Verification items for the finished model (mm, model axes). A direction names the side the tool comes from. Coordinates: 2 decimals unless noted, no trailing zeros. Write each loop counter-clockwise with the first axis right and the second up, starting at its lowest first coordinate (ties: lowest second). Pieces come first, ordered by that corner, then holes. Notation, with made-up numbers: (10.25, 74) -> (30.25, 74) arc R9 cw to (30.25, 86) -> close; hole circle Ø8 at (36, -1.75). An arc over 180 degrees is marked (long way). Answer in a Markdown table with one row per item.
```python
from build123d import *

# Parameters (mm, degrees)
SKETCH1_R                  = 40
SKETCH1_R_2                = 30
BOSS_EXTRUDE1_DEPTH        = 537.5
CUT_EXTRUDE1_START         = -25
SKETCH2_R                  = 55.029082457
SKETCH2_R_2                = 36.75
CUT_EXTRUDE1_DEPTH         = 3
SKETCH3_R                  = 40
SKETCH3_R_2                = 38
CUT_EXTRUDE2_DEPTH         = 25
CHAMFER1_SIZE              = 1
SKETCH4_R                  = 33.575067705
BOSS_EXTRUDE2_DEPTH        = 40
SKETCH5_R                  = 25
CUT_EXTRUDE3_DEPTH         = 6
SKETCH6_R                  = 21.5
CUT_EXTRUDE4_DEPTH         = 535.501870904
CHAMFER2_SIZE              = 1
SKETCH9_R                  = 30
CUT_EXTRUDE7_DEPTH         = 40
SKETCH10_R                 = 35
CUT_EXTRUDE8_DEPTH         = 7
M64X4_0_TAPPED_HOLE1_D     = 60
M64X4_0_TAPPED_HOLE1_DEPTH = 20
M64X4_0_TAPPED_HOLE1_TIP   = 18.025818571
CHAMFER3_SIZE              = 0.5
CHAMFER4_SIZE              = 0.5
SKETCH13_R                 = 40
CUT_EXTRUDE9_DEPTH         = 3
CHAMFER5_SIZE              = 1
CHAMFER7_SIZE              = 0.5
FILLET1_R                  = 0.5
M64X3_0_TAPPED_HOLE1_D     = 61
M64X3_0_TAPPED_HOLE1_DEPTH = 55
M64X3_0_TAPPED_HOLE1_TIP   = 18.32624888
CHAMFER8_SIZE              = 1


with BuildPart() as part:
    # Sketch1 → Boss-Extrude1 (new body)
    with BuildSketch(Plane(origin=(0, 0, 0), x_dir=(1, 0, 0), z_dir=(0, 1, 0))):
        with Locations(Location((0, 0, 0), (0, 0, 270))):
            Circle(SKETCH1_R)
        with Locations(Location((0, 0, 0), (0, 0, 270))):
            Circle(SKETCH1_R_2, mode=Mode.SUBTRACT)
    extrude(amount=BOSS_EXTRUDE1_DEPTH)

    # Sketch2 → Cut-Extrude1 (cut)
    with BuildSketch(Plane.XZ.offset(CUT_EXTRUDE1_START)):
        Circle(SKETCH2_R)
        with Locations(Location((0, 0, 0), (0, 0, 270))):
            Circle(SKETCH2_R_2, mode=Mode.SUBTRACT)
    extrude(amount=-CUT_EXTRUDE1_DEPTH, mode=Mode.SUBTRACT)

    # Sketch3 → Cut-Extrude2 (cut)
    with BuildSketch(Plane.XZ):
        with Locations(Location((0, 0, 0), (0, 0, 270))):
            Circle(SKETCH3_R)
        with Locations(Location((0, 0, 0), (0, 0, 270))):
            Circle(SKETCH3_R_2, mode=Mode.SUBTRACT)
    extrude(amount=-CUT_EXTRUDE2_DEPTH, mode=Mode.SUBTRACT)

    # Chamfer1
    chamfer1_edges = [part.edges().sort_by_distance(p)[0] for p in [
        (0, 0, 38),
        (0, 537.5, -40),
    ]]
    chamfer(chamfer1_edges, length=CHAMFER1_SIZE)

    # Sketch4 → Boss-Extrude2 (add)
    with BuildSketch(Plane(origin=(0, 537.5, 0), x_dir=(1, 0, 0), z_dir=(0, 1, 0))):
        Circle(SKETCH4_R)
    extrude(amount=-BOSS_EXTRUDE2_DEPTH)

    # Sketch5 → Cut-Extrude3 (cut)
    with BuildSketch(Plane(origin=(0, 537.5, 0), x_dir=(1, 0, 0), z_dir=(0, 1, 0))):
        with Locations(Location((0, 0, 0), (0, 0, 270))):
            Circle(SKETCH5_R)
    extrude(amount=-CUT_EXTRUDE3_DEPTH, mode=Mode.SUBTRACT)

    # Sketch6 → Cut-Extrude4 (cut, through all)
    with BuildSketch(Plane(origin=(0, 531.5, 0), x_dir=(1, 0, 0), z_dir=(0, 1, 0))):
        with Locations(Location((0, 0, 0), (0, 0, 270))):
            Circle(SKETCH6_R)
    extrude(amount=-CUT_EXTRUDE4_DEPTH, mode=Mode.SUBTRACT)

    # Chamfer2
    chamfer2_edges = [part.edges().sort_by_distance(p)[0] for p in [
        (0, 531.5, -21.5),
    ]]
    chamfer(chamfer2_edges, length=CHAMFER2_SIZE)

    # Sketch9 → Cut-Extrude7 (cut)
    with BuildSketch(Plane.XZ.offset(-497.5)):
        with Locations(Location((0, 0, 0), (0, 0, 90))):
            Circle(SKETCH9_R)
    extrude(amount=-CUT_EXTRUDE7_DEPTH, mode=Mode.SUBTRACT)

    # Sketch10 → Cut-Extrude8 (cut)
    with BuildSketch(Plane(origin=(0, 537.5, 0), x_dir=(1, 0, 0), z_dir=(0, 1, 0))):
        with Locations(Location((0, 0, 0), (0, 0, 270))):
            Circle(SKETCH10_R)
    extrude(amount=-CUT_EXTRUDE8_DEPTH, mode=Mode.SUBTRACT)

    # M64x4.0 Tapped Hole1
    with Locations(Plane(origin=(0, 530.5, 0), x_dir=(1, 0, 0), z_dir=(0, 1, 0))):
        with Locations((0, 0)):
            Hole(M64X4_0_TAPPED_HOLE1_D / 2, depth=M64X4_0_TAPPED_HOLE1_DEPTH)
            with Locations((0, 0, -(M64X4_0_TAPPED_HOLE1_DEPTH + M64X4_0_TAPPED_HOLE1_TIP / 2))):  # 118° drill point
                Cone(0, M64X4_0_TAPPED_HOLE1_D / 2, M64X4_0_TAPPED_HOLE1_TIP, mode=Mode.SUBTRACT)

    # Chamfer3
    chamfer3_edges = [part.edges().sort_by_distance(p)[0] for p in [
        (0, 537.5, -35),
    ]]
    chamfer(chamfer3_edges, length=CHAMFER3_SIZE)

    # Chamfer4
    chamfer4_edges = [part.edges().sort_by_distance(p)[0] for p in [
        (0, 530.5, -30),
    ]]
    chamfer(chamfer4_edges, length=CHAMFER4_SIZE)

    # Sketch13 → Cut-Extrude9 (cut)
    with BuildSketch(Plane.XZ):
        with Locations(Location((0, 0, 0), (0, 0, 270))):
            Circle(SKETCH13_R)
    extrude(amount=-CUT_EXTRUDE9_DEPTH, mode=Mode.SUBTRACT)

    # Chamfer5
    chamfer5_edges = [part.edges().sort_by_distance(p)[0] for p in [
        (0, 3, 38),
    ]]
    chamfer(chamfer5_edges, length=CHAMFER5_SIZE)

    # Chamfer7
    chamfer7_edges = [part.edges().sort_by_distance(p)[0] for p in [
        (0, 28, -40),
    ]]
    chamfer(chamfer7_edges, length=CHAMFER7_SIZE)

    # Fillet1
    fillet1_edges = [part.edges().sort_by_distance(p)[0] for p in [
        (0, 28, 36.75),
        (0, 25, 36.75),
    ]]
    fillet(fillet1_edges, radius=FILLET1_R)

    # M64x3.0 Tapped Hole1
    with Locations(Plane(origin=(0, 530.5, 0), x_dir=(1, 0, 0), z_dir=(0, 1, 0))):
        with Locations((0, 0)):
            Hole(M64X3_0_TAPPED_HOLE1_D / 2, depth=M64X3_0_TAPPED_HOLE1_DEPTH)
            with Locations((0, 0, -(M64X3_0_TAPPED_HOLE1_DEPTH + M64X3_0_TAPPED_HOLE1_TIP / 2))):  # 118° drill point
                Cone(0, M64X3_0_TAPPED_HOLE1_D / 2, M64X3_0_TAPPED_HOLE1_TIP, mode=Mode.SUBTRACT)

    # Chamfer8
    chamfer8_edges = [part.edges().sort_by_distance(p)[0] for p in [
        (30.5, 530.5, 0),
    ]]
    chamfer(chamfer8_edges, length=CHAMFER8_SIZE)


solid = part.part
```
1. Access from +Z, -Z, +X, -X, +Y, -Y to the whole of each face (thin tool, end or side, straight path). Record for faces 5 (the face through (28, 25, -25)), 6 (the face through (-39.05, 278.94, -8.67)), 7 (the face through (-21, 534, -28)).
Findings below:
| item | result |
|---|---|
| face 5 | none |
| face 6 | +Y, -Y |
| face 7 | +Y |
2. Go/stop test with flat-tipped pins: pin 1 (12 mm diameter, centred on y = 246.5, z = 13.5, fed in from +X); pin 2 (6 mm diameter, centred on y = 239, z = 2.5, fed in from +X); pin 3 (10 mm diameter, centred on y = 172, z = 22.5, fed in from +X). Record where each tip stops, or that it passes through.
Findings below:
| item | result |
|---|---|
| pin 1 | stops at x = 39.29 |
| pin 2 | stops at x = 40 |
| pin 3 | stops at x = 35.97 |
3. Material ranges on probe 1 along Z at (x, y) = (0, 186); probe 2 along X at (y, z) = (534, 0), recorded low to high. Write a range as from..to.
Findings below:
| item | result |
|---|---|
| probe 1 | z = -40..-30, 30..40 |
| probe 2 | x = -40..-35, 35..40 |
4. Release check for a two-part mould opening along X. For faces 1 (the face through (13, 530.5, -29)), 2 (the face through (24.204, 502.122, 18.559)), 3 (the face through (30.3, 3, 0.2)), 4 (the face through (-23.122, 14.353, 30.156)) record: released by +X, released by -X, zero draft, split by the parting line, or undercut.
Findings below:
| item | result |
|---|---|
| face 1 | undercut |
| face 2 | undercut |
| face 3 | zero draft |
| face 4 | split by the parting line |
5. Sectioned sample at A-A, the plane y = 467. Record the cut outline in (x, z), and give its area (3 significant figures).
Findings below:
| item | result |
|---|---|
| outline | circle Ø80 at (0, 0); hole circle Ø60 at (0, 0) |
| area | 2,200 mm² |
